```python
from build123d import *

# Parameters (mm, degrees)
SKETCH_1_R      = 5
EXTRUDE_1_DEPTH = 55


with BuildPart() as part:
    # 草图1 → 凸台-拉伸1 (new, symmetric)
    with BuildSketch(Plane.XY):
        Circle(SKETCH_1_R)
    extrude(amount=EXTRUDE_1_DEPTH, both=True)

    # 草图3 → M5x0.8 螺纹孔1 (revolve, cut)
    with BuildSketch(Plane(origin=(0, 0, 55), x_dir=(0, -1, 0), z_dir=(1, 0, 0))):
        Polygon((0, 0), (0, 13.6618073), (2.1, 12.4), (2.1, 0.425), (2.525, 0), align=None)
    m5x0_8_1 = revolve(axis=Axis((0, 0, 61.35), (0, 0, -1)), mode=Mode.SUBTRACT)

    # 镜向1: M5x0.8 螺纹孔1 across plane
    add(m5x0_8_1.mirror(Plane.XY), mode=Mode.SUBTRACT)


solid = part.part
```
The listing builds one solid part. Answer for the finished solid, in the listing's coordinates (mm). A direction names the side the tool comes from. Round coordinates to 2 decimals unless told otherwise and drop trailing zeros. Loops run counter-clockwise (first coordinate to the right, second up) from the corner with the lowest first, then second, coordinate; pieces in that order, holes last.
Q1. Which of the six approach directions +Z, -Z, +X, -X, +Y, -Y give full straight-line access (tool end or side, diameter ignored) to faces 1 (the face through (-0.631, -2.003, 48.671)), 2 (the face through (-0.631, -2.003, -48.671)), 3 (the face through (2, -2, 55))?
Q2. Section A-A, the plane y = 4 is taken. Determine the outline of the cut face in (x, z).
Q3. For a pull along Y with two mould halves and no side action, classify faces 4 (the face through (-0.11, -0.35, 41.56)), 5 (the face through (-1.08, -4.88, 0.77)), 6 (the face through (2, -2, -55)) as released by +Y, released by -Y, zero draft, split by the parting line, or undercut.
Q4. Given pin 1 Ø4 at (x, y) = (0, 0) entering from +Z; pin 2 Ø5 at (x, y) = (0, 0) entering from -Z (3 decimals), each flat-ended and moving along its own axis, determine where each tip first touches the part or whether it passes through.
Q5. Section C-C, the plane z = -27 is taken. Determine the outline of the cut face in (x, y), then the cut area to 3 significant figures.
Q6. Find the intervals of material crossed by line 1 (Y direction, x = 0, z = 49.75); line 2 (X direction, y = -0.75, z = -48); line 3 (X direction, y = 0.25, z = 36.5), in increasing order.
Completed:
1. face 1: +Z
1. face 2: -Z
1. face 3: +Z, +X, -X, +Y, -Y
2. outline: (-3, -55) - (3, -55) - (3, 55) - (-3, 55) - close
3. face 4: undercut
3. face 5: split by the parting line
3. face 6: zero draft
4. pin 1: stops at z = 42.54
4. pin 2: stops at z = -54.975
5. outline: circle Ø10 at (0, 0)
5. area: 78.5 mm2
6. line 1: y = -5 to -2.1, 2.1 to 5
6. line 2: x = -4.94 to -1.96, 1.96 to 4.94
6. line 3: x = -4.99 to 4.99
